from build123d import *

# Parameters (mm, degrees)
F_9_16_0_5625_DIAMETER_HOLE1_D = 14.2875
F_1_2_13_TAPPED_HOLE1_D        = 10.71626
EXTRUDE1_START                 = 55.626
SKETCH8_W                      = 36.576
SKETCH8_H                      = 25.4
EXTRUDE1_DEPTH                 = 4.6863
EXTRUDE2_REACH                 = 184.013
EXTRUDE2_END_RADIUS            = 46.865
FILLET1_R                      = 3


with BuildPart() as part:
    # Sketch1 → Revolve1 (revolve)
    with BuildSketch(Plane.XY):
        Polygon((-65.8622, 50.618781854), (-65.8622, 60.0705), (-59.5122, 60.3123), (-12.7, 60.3123), (-12.7, 88.9), (0, 88.9), (0, 0), (-18.159, 0), (-18.159, 46.865), (-33.909, 46.865), (-33.909, 50.00625), (-58.7756, 50.00625), (-58.7756, 53.0098), (-61.8236, 53.0098), (-61.8236, 50.00625), (-63.5762, 50.00625), align=None)
    revolve(axis=Axis((0, 0, 0), (-1, 0, 0)))

    # 9/16 (0.5625) Diameter Hole1 (through all)
    with Locations(Plane(origin=(0, 0, 0), x_dir=(0, 0, -1), z_dir=(1, 0, 0))):
        with Locations((-51.6382, 51.6382), (51.6382, 51.6382), (-36.5252, -63.246), (36.5252, -63.246)):
            Hole(F_9_16_0_5625_DIAMETER_HOLE1_D / 2)

    # 1/2-13 Tapped Hole1 (through all)
    with Locations(Plane(origin=(0, 0, 0), x_dir=(0, 0, -1), z_dir=(1, 0, 0))):
        with Locations((-73.025, 0), (73.025, 0)):
            Hole(F_1_2_13_TAPPED_HOLE1_D / 2)

    # Sketch8 → Extrude1 (cut)
    with BuildSketch(Plane(origin=(0, 0, 0), x_dir=(1, 0, 0), z_dir=(0, 1, 0)).offset(EXTRUDE1_START)):
        with Locations((-30.988, 0)):
            Rectangle(SKETCH8_W, SKETCH8_H)
    extrude(amount=EXTRUDE1_DEPTH, mode=Mode.SUBTRACT)

    # Extrude2: up to this cylinder (the profile starts outside it)
    extrude2_end = Plane(origin=(-18.090047, 0, 0), z_dir=(1, 0, 0)) * Cylinder(EXTRUDE2_END_RADIUS, 462.756, mode=Mode.PRIVATE)
    # Sketch9 → Extrude2 (cut, up to the surface)
    with BuildSketch(Plane(origin=(0, 55.626, 0), x_dir=(1, 0, 0), z_dir=(0, 1, 0)), mode=Mode.PRIVATE) as extrude2_sk1:
        with BuildLine():
            Line((-12.7, 12.7), (-12.7, -12.7))
            ThreePointArc((-12.7, -12.7), (-25.4, 0), (-12.7, 12.7))
        make_face()
    extrude2_tool1 = extrude(extrude2_sk1.sketch, amount=-EXTRUDE2_REACH, mode=Mode.PRIVATE) - extrude2_end
    add(extrude2_tool1.solids().sort_by_distance((-18.090047, 55.626, 0))[0], mode=Mode.SUBTRACT)

    # Fillet1
    fillet1_edges = [part.edges().sort_by_distance(p)[0] for p in [
        (-49.276, 57.293008189, 12.7),
        (-49.276, 57.293008189, -12.7),
    ]]
    fillet(fillet1_edges, radius=FILLET1_R)


solid = part.part
Could you check a few things on this model? Use its own coordinates, in mm. A direction names the side the tool comes from. Coordinates: 2 decimals unless noted, no trailing zeros. Order: outer loops, then holes, each group sorted by start corner. A loop starts at its lowest first (then second) coordinate and runs counter-clockwise, first axis right, second up.
Q1. Suppose I cut it at D-D on x = -15. Please give me the cut outline in (y, z) (3 decimals), and give its area (3 significant figures).
Q2. Suppose I cut it at A-A on z = 76. Please give me the cut outline in (x, y).
Q3. Suppose I cut it at B-B on x = -53. Please give me the cut outline in (y, z).
Q4. Thinking about a two-plate mould opening in Z: for faces 4 (the cylindrical face through (-26.14, 44.7, -14.08)), 5 (the cylindrical face through (-15.391, 46.865, -0.18)), 6 (the cylindrical face through (-6.261, 84.795, -26.703)), 7 (the flat face through (-65.862, 27, 44)), which applies, released by +Z, released by -Z, zero draft, split by the parting line, or undercut?
Q5. Will these pins go through, and if not, where does the flat tip stop? pin 1 (6 mm diameter, centred on x = -41.5, y = 13.5, fed in from +Z); pin 2 (1 mm diameter, centred on y = 2, z = 28, fed in from -X); pin 3 (13 mm diameter, centred on y = 51.64, z = 51.64, fed in from -X); pin 4 (6 mm diameter, centred on x = -8.5, z = 12.5, fed in from +Y).
Q6. Please list where these lines run through material, in increasing order: L1, parallel to Z at x = -27, y = 0 (3 decimals); L2, parallel to Y at x = -28, z = 0 (3 decimals); L3, parallel to X at y = 65.5, z = 15.
Q7. Suppose I cut it at C-C on y = 0. Give the number of separate pieces and of enclosed holes in the cut face, and give its area (3 significant figures).
Q8. Which directions (+Z, -Z, +X, -X, +Y, -Y) give clear straight access to the entire face, cutting with the end or side of a thin tool? Please do faces 1 (the cylindrical face through (-60.321, 50.562, -15.923)), 2 (the cylindrical face through (-6.439, -2.052, 77.975)), 3 (the cylindrical face through (-46.516, -10.84, 48.817)).
Answer:
1. outline: (45.17, -12.49) arc R46.865 ccw to (45.17, 12.49) - (55.626, 12.49) - (55.626, 12.7) - (58.96, 12.7) arc R60.312 ccw (long way) to (58.96, -12.7) - (55.626, -12.7) - (55.626, -12.49) - close
1. area: 11,100 mm2
2. outline: (-12.7, -46.12) - (0, -46.12) - (0, -4.46) - (-12.7, -4.46) - close; (-12.7, 4.46) - (0, 4.46) - (0, 46.12) - (-12.7, 46.12) - close
3. outline: circle Ø120.62 at (0, 0); hole circle Ø100.01 at (0, 0)
4. face 4: undercut
4. face 5: undercut
4. face 6: split by the parting line
4. face 7: zero draft
5. pin 1: stops at z = 59.39
5. pin 2: stops at x = -18.16
5. pin 3: passes through
5. pin 4: stops at y = 88.39
6. L1: z = -60.312 to -46.865, 46.865 to 60.312
6. L2: y = -60.312 to -46.865, 46.865 to 55.626
6. L3: x = -12.7 to 0
7. separate pieces: 3
7. enclosed holes: 0
7. area: 3,710 mm2
8. face 1: none
8. face 2: +X, -X
8. face 3: -X
